Can you work these out from the model? Positions are in its coordinate system, mm. A direction names the side the tool comes from. Round coordinates to 2 decimals unless told otherwise and drop trailing zeros. Write each loop counter-clockwise with the first axis right and the second up, starting at its lowest first coordinate (ties: lowest second). Pieces come first, ordered by that corner, then holes. Notation, with made-up numbers: (44.25, -17.5) - (98.25, -17.5) arc R14 cw to (98.25, -4.5) - close; hole circle Ø10 at (13, 85). An arc over 180 degrees is marked (long way). One line per item, written item: value. Start each with the question number.
(1) I want a section at C-C on z = 14.5. List the corners of the cut face in (x, y) for me.
(2) If I drill on L1, parallel to Z at x = 8.25, y = -6.75; L2, parallel to Y at x = -4.5, z = -3; L3, parallel to X at y = -7, z = -30, over which ranges is the centre line in solid material (lowest first)? Write a range as from..to.
(3) I want a section at A-A on x = 6.25. List the corners of the cut face in (y, z) for me.
(4) I want a section at B-B on y = -1.75. List the corners of the cut face in (x, z) for me.
(5) I want a section at D-D on x = 11.75. List the corners of the cut face in (y, z) for me.
(6) On a 3-axis mill with a long thin cutter (end or side, diameter ignored), from which of +Z, -Z, +X, -X, +Y, -Y can I reach the whole of each face in a straight line? I mean faces 1 (the face through (6, 7, 0)), 2 (the face through (6, 7, 3)), 3 (the face through (8.605, 8.365, 1.479)). Say none if no direction works.
(7) I'm going to push flat-ended pins straight in: pin 1 Ø12 at (y, z) = (-5.5, 8) entering from +X; pin 2 Ø1 at (x, y) = (5, 8.5) entering from -Z; pin 3 Ø3 at (x, z) = (-9, -13) entering from +Y. Where does each tip first touch, or does it pass through?
from build123d import *

# Parameters (mm, degrees)
BOSS_EXTRUDE1_DEPTH      = 20
BOSS_EXTRUDE1_DEPTH_BACK = 33
SKETCH1_R                = 9
BOSS_EXTRUDE2_DEPTH      = 3


with BuildPart() as part:
    # Sketch1 → Boss-Extrude1 (new, two sides: drawn at the far end of the back side and taken through both)
    with BuildSketch(Plane.XY.offset(-BOSS_EXTRUDE1_DEPTH_BACK)):
        Circle(SKETCH1_R)
    extrude(amount=BOSS_EXTRUDE1_DEPTH + BOSS_EXTRUDE1_DEPTH_BACK)

    # Sketch2 → Boss-Extrude2 (add)
    with BuildSketch(Plane.XY):
        Polygon((9.738398553, -9.857159511), (13.405749822, 3.505120784), (3.667351269, 13.362280294), (-9.738398553, 9.857159511), (-13.405749822, -3.505120784), (-3.667351269, -13.362280294), align=None)
    extrude(amount=BOSS_EXTRUDE2_DEPTH)


solid = part.part
Established:
1. outline: circle Ø18 at (0, 0)
2. L1: 0..3
2. L2: -7.79..7.79
2. L3: -5.66..5.66
3. outline: (-10.77, 0) - (-6.48, 0) - (-6.48, -33) - (6.48, -33) - (6.48, 0) - (10.75, 0) - (10.75, 3) - (6.48, 3) - (6.48, 20) - (-6.48, 20) - (-6.48, 3) - (-10.77, 3) - close
4. outline: (-12.92, 0) - (-8.83, 0) - (-8.83, -33) - (8.83, -33) - (8.83, 0) - (11.96, 0) - (11.96, 3) - (8.83, 3) - (8.83, 20) - (-8.83, 20) - (-8.83, 3) - (-12.92, 3) - close
5. outline: (-2.53, 0) - (5.18, 0) - (5.18, 3) - (-2.53, 3) - close
6. face 1: -Z
6. face 2: +Z
6. face 3: +Z, -Z, +X, +Y
7. pin 1: x = 11.84
7. pin 2: z = 0
7. pin 3: y = 4.97
